Model file for the job. Use its own axes, mm. Face numbers are marked on the shaded views. A direction names the side the tool comes from. Coordinates: 2 decimals unless noted, no trailing zeros. Write each loop counter-clockwise with the first axis right and the second up, starting at its lowest first coordinate (ties: lowest second). Pieces come first, ordered by that corner, then holes. Notation, with made-up numbers: M 39,16.5 L 59,16.5 A29 cw 59,49.5 Z; hole C 5.5,-24 d1. An arc over 180 degrees is marked long. One line per question, with ' | ' between items. Start each with the question number.
(1) Wall check: probe 1 along X at (y, z) = (-33, -7); probe 2 along X at (y, z) = (51.5, -3); probe 3 along X at (y, z) = (-33, -17.5). Give the ranges that are in metal, low to high.
(2) Cut at A-A (y = 18). Write the cut outline in (x, z), plus the area to 3 significant figures.
(3) Two-plate mould, pull along X, no slides. Class the marked faces 4, 5 and 6: +X half, -X half, draft (parallel to the pull), parting line (faces both ways), or undercut.
(4) Cut at D-D (y = 51.5). Write the cut outline in (x, z).
(5) Flat gauge pins, fed straight in: pin 1 Ø15 at (y, z) = (30.5, -8.5) entering from -X; pin 2 Ø25 at (x, z) = (-62, 12.5) entering from +Y; pin 3 Ø8 at (x, z) = (64.5, 3) entering from +Y. Where does each tip first touch, or does it go through?
(6) Tool access for the marked faces 1, 2 and 3: list every direction of +Z, -Z, +X, -X, +Y, -Y with a clear straight run to the whole face (end or side of a thin tool).
(7) Cut at B-B (x = -77.5). Write the cut outline in (y, z).
(8) Cut at C-C (z = 2.5). Write the cut outline in (x, y), plus the area to 3 significant figures.
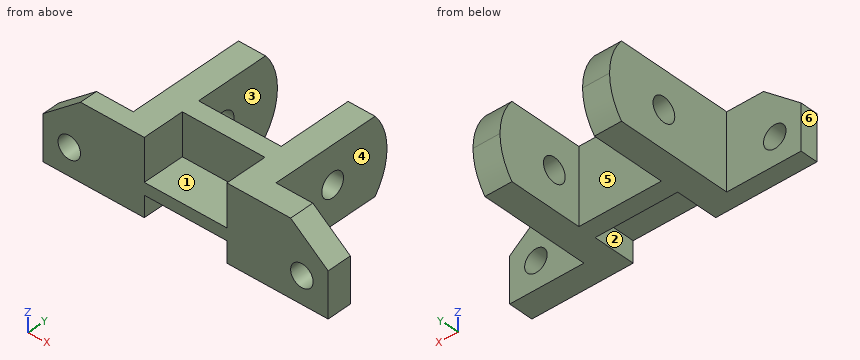
from build123d import *
from OCP.BRepFilletAPI import BRepFilletAPI_MakeChamfer

# Parameters (mm, degrees)
BRACKET_BODY_DEPTH                           = 25
UPRIGHT_ROUNDS_AND_PIN_HOLE_SKETCH_R         = 8
UPRIGHT_ROUNDS_AND_PIN_HOLE_16_DEPTH         = 120
FLANGE_CORNER_CHAMFERS_SIZE                  = 20
FLANGE_CORNER_CHAMFERS_SIZE2                 = 25
MOUNTING_HOLES_AND_RELIEF_SKETCH_R           = 7.5
MOUNTING_HOLES_AND_RELIEF_SKETCH_W           = 55
MOUNTING_HOLES_AND_RELIEF_SKETCH_H           = 28
MOUNTING_HOLES_AND_RELIEF_SKETCH_H_2         = 14
MOUNTING_HOLES_2X_15_AND_CENTRE_RELIEF_DEPTH = 28


with BuildPart() as part:
    # Bracket Side Profile Sketch → Bracket Body (new, symmetric)
    with BuildSketch(Plane.XY):
        Polygon((-95, -28.245219348), (-95, -40), (95, -40), (95, -23.642294713), (45.5, -23.642294713), (45.5, 58), (27.5, 58), (27.5, 0), (-27.5, 0), (-27.5, 58), (-45.5, 58), (-45.5, -28.245219348), align=None)
    extrude(amount=BRACKET_BODY_DEPTH, both=True)

    # Upright Rounds and Pin Hole Sketch → Upright Rounds and Pin Hole Ø16 (cut)
    with BuildSketch(Plane(origin=(45.5, 0, 0), x_dir=(0, 0, -1), z_dir=(1, 0, 0))):
        with BuildLine():
            Line((-25, 58), (-25, 49.224989992))
            ThreePointArc((-25, 49.224989992), (-13.24764886, 55.74254628), (-1.3e-08, 58))
            Line((-1.3e-08, 58), (-25, 58))
        make_face()
        Polygon((-25, 66.800794381), (-25, 58), (-1.3e-08, 58), (25, 58), (25, 66.800794381), align=None)
        with BuildLine():
            Line((25, 58), (-1.3e-08, 58))
            ThreePointArc((-1.3e-08, 58), (13.247648848, 55.742546284), (25, 49.224989992))
            Line((25, 49.224989992), (25, 58))
        make_face()
        with Locations((0, 18)):
            Circle(UPRIGHT_ROUNDS_AND_PIN_HOLE_SKETCH_R)
    extrude(amount=-UPRIGHT_ROUNDS_AND_PIN_HOLE_16_DEPTH, mode=Mode.SUBTRACT)

    # Flange Corner Chamfers: one chamfer whose edges measure the first distance from different faces: ONE call of the kernel's chamfer builder (chamfer() names one face for all edges)
    flange_corner_chamfers_edges_1 = [part.edges().sort_by_distance(p)[0] for p in [
        (95, -31.821147357, 25),
    ]]
    flange_corner_chamfers_side_1 = [part.faces().sort_by_distance(p)[0] for p in [
        (95, -31.821147357, 0),
    ]]
    flange_corner_chamfers_edges_2 = [part.edges().sort_by_distance(p)[0] for p in [
        (-95, -34.122609674, 25),
    ]]
    flange_corner_chamfers_side_2 = [part.faces().sort_by_distance(p)[0] for p in [
        (-95, -34.122609674, 0),
    ]]
    flange_corner_chamfers = BRepFilletAPI_MakeChamfer(part.part.solid().wrapped)
    for e in flange_corner_chamfers_edges_1:
        flange_corner_chamfers.Add(FLANGE_CORNER_CHAMFERS_SIZE, FLANGE_CORNER_CHAMFERS_SIZE2, e.wrapped, flange_corner_chamfers_side_1[0].wrapped)  # the first distance lies on this face
    for e in flange_corner_chamfers_edges_2:
        flange_corner_chamfers.Add(FLANGE_CORNER_CHAMFERS_SIZE, FLANGE_CORNER_CHAMFERS_SIZE2, e.wrapped, flange_corner_chamfers_side_2[0].wrapped)  # the first distance lies on this face
    add(Compound.cast(flange_corner_chamfers.Shape()), mode=Mode.REPLACE)

    # Mounting Holes and Relief Sketch → Mounting Holes 2xØ15 and Centre Relief (cut)
    with BuildSketch(Plane.XZ.offset(40)):
        with Locations(Location((-77.5, -7, 0), (0, 0, 270))):
            Circle(MOUNTING_HOLES_AND_RELIEF_SKETCH_R)
        with Locations(Location((77.5, -7, 0), (0, 0, 270))):
            Circle(MOUNTING_HOLES_AND_RELIEF_SKETCH_R)
        with Locations((0, 11)):
            Rectangle(MOUNTING_HOLES_AND_RELIEF_SKETCH_W, MOUNTING_HOLES_AND_RELIEF_SKETCH_H)
        with Locations((0, -18)):
            Rectangle(MOUNTING_HOLES_AND_RELIEF_SKETCH_W, MOUNTING_HOLES_AND_RELIEF_SKETCH_H_2)
    extrude(amount=-MOUNTING_HOLES_2X_15_AND_CENTRE_RELIEF_DEPTH, mode=Mode.SUBTRACT)


solid = part.part
Filled in:
1) probe 1: -95 to -85, -70 to 70, 85 to 95 | probe 2: -45.5 to -27.5, 27.5 to 45.5 | probe 3: -95 to -27.5, 27.5 to 95
2) outline: M -45.5,-25 L -27.5,-25 L -27.5,-8 L -45.5,-8 Z; M -45.5,8 L -27.5,8 L -27.5,25 L -45.5,25 Z; M 27.5,-25 L 45.5,-25 L 45.5,-8 L 27.5,-8 Z; M 27.5,8 L 45.5,8 L 45.5,25 L 27.5,25 Z | area: 1,220 mm²
3) face 4: +X half | face 5: undercut | face 6: -X half
4) outline: M -45.5,-21.86 L -27.5,-21.86 L -27.5,21.86 L -45.5,21.86 Z; M 27.5,-21.86 L 45.5,-21.86 L 45.5,21.86 L 27.5,21.86 Z
5) pin 1: x = -45.5 | pin 2: y = -28.25 | pin 3: y = -23.64
6) face 1: +Z, -Y | face 2: -Z, -Y | face 3: +Z, -Z, +Y
7) outline: M -40,-25 L -28.25,-25 L -28.25,-14.5 L -40,-14.5 Z; M -40,0.5 L -28.25,0.5 L -28.25,19 L -40,19 Z
8) outline: M -95,-40 L -27.5,-40 L -27.5,-12 L 27.5,-12 L 27.5,-40 L 95,-40 L 95,-23.64 L 45.5,-23.64 L 45.5,10.4 L 27.5,10.4 L 27.5,0 L -27.5,0 L -27.5,10.4 L -45.5,10.4 L -45.5,-28.25 L -95,-28.25 Z; M -45.5,25.6 L -27.5,25.6 L -27.5,57.92 L -45.5,57.92 Z; M 27.5,25.6 L 45.5,25.6 L 45.5,57.92 L 27.5,57.92 Z | area: 5,030 mm²
